The listing builds one solid part. Answer for the finished solid, in the listing's coordinates (mm). A direction names the side the tool comes from. Coordinates: 2 decimals unless noted, no trailing zeros. Write each loop counter-clockwise with the first axis right and the second up, starting at its lowest first coordinate (ties: lowest second). Pieces come first, ordered by that corner, then holes. Notation, with made-up numbers: M 14.25,23 L 33.25,23 A21 ccw 33.25,38 Z; hole C 17,66.25 d7. An arc over 180 degrees is marked long. Answer as CSV lines item,"result".
```python
from build123d import *

# Parameters (mm, degrees)
BOSS_EXTRUDE1_DEPTH     = 205
FILLET1_R               = 5
SKETCH2_R               = 45
CUT_EXTRUDE1_DEPTH      = 582.424113707
CUT_EXTRUDE2_DEPTH      = 380.537876952
CUT_EXTRUDE3_DEPTH      = 5
CUT_EXTRUDE3_DEPTH_BACK = 354.691405041
SKETCH5_R               = 232
BOSS_EXTRUDE2_DEPTH     = 30
CUT_EXTRUDE4_DEPTH      = 53.1
M8_TAPPED_HOLE1_D       = 6.8
M8_TAPPED_HOLE1_DEPTH   = 20.207073895
M8_TAPPED_HOLE1_TIP     = 2.042926105


with BuildPart() as part:
    # Sketch1 → Boss-Extrude1 (new body)
    with BuildSketch(Plane.XY):
        with BuildLine():
            Line((-227.111967186, 47), (-223, 0))
            Line((-223, 0), (282, 0))
            Line((282, 0), (282, 35))
            Line((282, 35), (260, 35))
            Line((260, 35), (260, 30))
            Line((260, 30), (190, 30))
            Line((190, 30), (190, 150))
            Line((190, 150), (107.739268607, 150))
            ThreePointArc((107.739268607, 150), (106.373112603, 149.134239248), (105, 148.279554695))
            Line((105, 148.279554695), (105, 30))
            Line((105, 30), (-105, 30))
            Line((-105, 30), (-105, 148.279554695))
            ThreePointArc((-105, 148.279554695), (-106.373112603, 149.134239248), (-107.739268607, 150))
            Line((-107.739268607, 150), (-151, 150))
            Line((-151, 150), (-151, 30))
            Line((-151, 30), (-191, 30))
            Line((-191, 30), (-191, 59))
            Line((-191, 59), (-241, 59))
            Line((-241, 59), (-241, 47))
            Line((-241, 47), (-227.111967186, 47))
        make_face()
    extrude(amount=-BOSS_EXTRUDE1_DEPTH)

    # Fillet1
    fillet1_edges = [part.edges().sort_by_distance(p)[0] for p in [
        (-105, 30, -102.5),
        (105, 30, -102.5),
    ]]
    fillet(fillet1_edges, radius=FILLET1_R)

    # Sketch2 → Cut-Extrude1 (cut, through all)
    with BuildSketch(Plane(origin=(282, 0, 0), x_dir=(0, 0, -1), z_dir=(1, 0, 0))):
        with Locations((102.5, 90)):
            Circle(SKETCH2_R)
    extrude(amount=-CUT_EXTRUDE1_DEPTH, mode=Mode.SUBTRACT)

    # Sketch3 → Cut-Revolve1 (revolve, cut)
    with BuildSketch(Plane(origin=(147.5, 0, 0), x_dir=(0, 0, -1), z_dir=(1, 0, 0)), mode=Mode.PRIVATE) as cut_revolve1_sk:
        Polygon((0, 95.9), (0, 90), (90, 90), (90, 95), align=None)
    revolve(cut_revolve1_sk.sketch.rotate(Axis((147.5, 90, -102.5), (0, 0, 1)), 136.455003644), axis=Axis((147.5, 90, -102.5), (0, 0, 1)), mode=Mode.SUBTRACT)

    # Sketch4 → Cut-Extrude2 (cut, through all)
    with BuildSketch(Plane(origin=(0, 0, -205), x_dir=(-1, 0, 0), z_dir=(0, 0, -1))):
        Polygon((-120, 150), (-105, 135), (-105, 150), align=None)
        Polygon((105, 150), (120, 150), (105, 135), align=None)
    extrude(amount=-CUT_EXTRUDE2_DEPTH, mode=Mode.SUBTRACT)

    # Sketch5 → Cut-Extrude3 (cut, two sides: drawn at the far end of the back side and taken through both)
    with BuildSketch(Plane(origin=(0, 0, -53.1), x_dir=(-1, 0, 0), z_dir=(0, 0, -1)).offset(-CUT_EXTRUDE3_DEPTH_BACK)):
        with Locations((0, 318.5)):
            Circle(SKETCH5_R)
    extrude(amount=CUT_EXTRUDE3_DEPTH + CUT_EXTRUDE3_DEPTH_BACK, mode=Mode.SUBTRACT)

    # Sketch6 → Boss-Extrude2 (add)
    with BuildSketch(Plane(origin=(0, 0, -205), x_dir=(-1, 0, 0), z_dir=(0, 0, -1))):
        Polygon((-282, 0), (223, 0), (227.111967186, 47), (241, 47), (241, 59), (191, 59), (191, 30), (-260, 30), (-260, 35), (-282, 35), align=None)
    extrude(amount=BOSS_EXTRUDE2_DEPTH)

    # Sketch7 → Cut-Extrude4 (cut)
    with BuildSketch(Plane.XY):
        Polygon((-151, 30), (-151, 146.183263941), (-120, 150), (-105, 135), (-105, 35), (-100, 30), align=None)
        Polygon((190, 150), (190, 30), (100, 30), (105, 35), (105, 135), (120, 150), align=None)
    extrude(amount=-CUT_EXTRUDE4_DEPTH, mode=Mode.SUBTRACT)

    # M8 Tapped Hole1
    with Locations(Plane(origin=(0, 59, 0), x_dir=(1, 0, 0), z_dir=(0, 1, 0))):
        with Locations((271, 29.3636836), (271, 219.953225124), (-219.303225542, 219.998090208), (-219.303225542, 29.3636836)):
            Hole(M8_TAPPED_HOLE1_D / 2, depth=M8_TAPPED_HOLE1_DEPTH)
            with Locations((0, 0, -(M8_TAPPED_HOLE1_DEPTH + M8_TAPPED_HOLE1_TIP / 2))):  # 118° drill point
                Cone(0, M8_TAPPED_HOLE1_D / 2, M8_TAPPED_HOLE1_TIP, mode=Mode.SUBTRACT)


solid = part.part
```
Q1. Find section B-B (y = 70). Give the vertices of the cut face in (x, z), and give its area (3 significant figures).
Output:
outline,"M -151,-205 L -105,-205 L -105,-142.81 L -151,-142.81 Z; M -151,-62.19 L -105,-62.19 L -105,-53.1 L -151,-53.1 Z; M 105,-205 L 190,-205 L 190,-142.81 L 105,-142.81 Z; M 105,-62.19 L 190,-62.19 L 190,-53.1 L 105,-53.1 Z"
area,"9,340 mm2"
Q2. Find section D-D (x = -26.5). Give the vertices of the cut face in (y, z), and give its area (3 significant figures).
Output:
outline,"M 0,-235 L 30,-235 L 30,0 L 0,0 Z"
area,"7,050 mm2"
Q3. The mould has two halves that part along X. Classify faces 1 (the flat face through (-241, 53, -175)), 2 (the flat face through (-113, 143, -133)), 3 (the flat face through (33, 0, -116)): pulls with the +X half, pulls with the -X half, needs draft (parallel to the pull), parting line crosses it, or undercut.
Output:
face 1,"pulls with the -X half"
face 2,"undercut"
face 3,"needs draft"
Q4. Find section C-C (z = -78.5). Count the separate pieces of the cut face and the enclosed holes in it, and give its area (3 significant figures).
Output:
separate pieces,"3"
enclosed holes,"0"
area,"21,700 mm2"
Q5. Find section A-A (z = -168). Give the vertices of the cut face in (x, y), and give its area (3 significant figures).
Output:
outline,"M -241,47 L -227.11,47 L -223,0 L 282,0 L 282,35 L 260,35 L 260,30 L 190,30 L 190,150 L 120,150 L 105,135 L 105,35 A5 cw 100,30 L -100,30 A5 cw -105,35 L -105,135 L -120,150 L -151,150 L -151,30 L -191,30 L -191,59 L -241,59 Z"
area,"32,000 mm2"
Q6. Straight lines are drawn through the part: line 1 (X direction, y = 91, z = -196); line 2 (X direction, y = 58, z = -138); line 3 (Y direction, x = 167, z = -102.5). For each, find the intervals that lie inside material, in ascending order.
Output:
line 1,"-151 to -105, 105 to 190"
line 2,"-241 to -191, -151 to -105, 105 to 190"
line 3,"0 to 45, 135 to 150"
Q7. Flat-ended cylindrical pins translate along their axes: pin 1 Ø3 at (y, z) = (130.5, -58) entering from -X; pin 2 Ø10 at (x, y) = (165, 49.5) entering from +Z; pin 3 Ø4 at (x, z) = (-237.5, -44.5) entering from -Y. Find the tip coordinate at first contact, or state that the pin passes through.
Output:
pin 1,"x = -151"
pin 2,"z = -53.1"
pin 3,"y = 47"
Q8. For faces 4 (the flat face through (113, 143, -133)), 5 (the flat face through (17, 17, 0)), 6 (the flat face through (-216, 59, -184)), 7 (the flat face through (-234, 47, -44)), 8 (the flat face through (271, 35, -116)), determine the directions among +Z, -Z, +X, -X, +Y, -Y from which every point of the face is accessible in a straight line to the end or side of a thin tool.
Output:
face 4,"+Z, -Z, +Y"
face 5,"+Z, +X, -X, +Y, -Y"
face 6,"+Z, -Z, -X, +Y"
face 7,"+Z, -Z, -X, -Y"
face 8,"+Z, -Z, +X, +Y"
